Here's how the part is built. I have some questions about the finished solid (model axes, mm). A direction names the side the tool comes from. Give positions to 0.01 mm unless a question says otherwise; leave off trailing zeros. Loops run counter-clockwise (first coordinate to the right, second up) from the corner with the lowest first, then second, coordinate; pieces in that order, holes last. Notation, with made-up numbers: M 58,56.25 L 108,56.25 A20 ccw 108,66.25 Z; hole C 0.25,9.5 d2. An arc over 180 degrees is marked long. Answer as CSV lines item,"result". Start each with the question number.
Item 1: For faces 1 (the flat face through (4.661, 49, 25)), 2 (the flat face through (54, 10, 15)), 3 (the flat face through (100, 5, 15)), which set-ups out of +Z, -Z, +X, -X, +Y, -Y let a thin tool reach every point of the face, with its end or its side?
Item 2: I want a section at B-B on z = 12.5. List the corners of the cut face in (x, y) for me, plus the area to 3 significant figures.
Item 3: I want a section at C-C on z = 5. List the corners of the cut face in (x, y) for me.
Item 4: If we mould it in two halves opening along Z, with no side actions, what happens to faces 4 (the flat face through (31, 9, 30)), 5 (the flat face through (6, 54, 11)), 6 (the cylindrical face through (4.023, 75.483, 12.24)), 7 (the cylindrical face through (4.023, 37.548, 12.066))? For each: released by +Z, released by -Z, zero draft, split by the parting line, or undercut.
Item 5: Will these pins go through, and if not, where does the flat tip stop? P1, Ø3, axis at y = 54, z = 25, coming from the +X side; P2, Ø1.1, axis at x = 5.5, y = 44, coming from the +Z side; P3, Ø9, axis at y = 33.5, z = 8.5, coming from the +X side; P4, Ø1, axis at x = 46.5, z = 9, coming from the -Y side.
Item 6: I want a section at D-D on y = 39.5. List the corners of the cut face in (x, z) for me, plus the area to 3 significant figures.
Item 7: If I drill on line 1 along Y through (x, z) = (4.05, 12.5); line 2 along Y through (x, z) = (21.5, 24); line 3 along X through (y, z) = (72.5, 5.5), over which ranges is the centre line in solid material (lowest first)? Write a range as from..to.
Item 8: I want a section at A-A on y = 73.5. List the corners of the cut face in (x, z) for me, plus the area to 3 significant figures.
from build123d import *

# Parameters (mm, degrees)
BOSS_EXTRUDE1_DEPTH = 30
SKETCH2_R           = 2
CUT_EXTRUDE1_DEPTH  = 145.568322948
CHAMFER1_SIZE       = 2.1
SKETCH3_W           = 2.678240958
SKETCH3_H           = 39.075972863
CUT_EXTRUDE2_DEPTH  = 10


with BuildPart() as part:
    # Sketch1 → Boss-Extrude1 (new body)
    with BuildSketch(Plane.XY):
        Polygon((0, 0), (100, 0), (100, 10), (6, 10), (6, 100), (0, 100), align=None)
    extrude(amount=BOSS_EXTRUDE1_DEPTH)

    # Sketch2 → Cut-Extrude1 (cut, through all)
    with BuildSketch(Plane.ZY):
        with Locations((12.5, 73.5)):
            Circle(SKETCH2_R)
        with Locations((12.5, 39.5)):
            Circle(SKETCH2_R)
    extrude(amount=-CUT_EXTRUDE1_DEPTH, mode=Mode.SUBTRACT)

    # Chamfer1
    chamfer1_edges = [part.edges().sort_by_distance(p)[0] for p in [
        (0, 73.5, 10.5),
        (0, 39.5, 10.5),
    ]]
    chamfer(chamfer1_edges, length=CHAMFER1_SIZE)

    # Sketch3 → Cut-Extrude2 (cut)
    with BuildSketch(Plane.XY.offset(30)):
        with Locations((6, 49.716029753)):
            Rectangle(SKETCH3_W, SKETCH3_H)
    extrude(amount=-CUT_EXTRUDE2_DEPTH, mode=Mode.SUBTRACT)


solid = part.part
Result:
1,face 1,"+Z, +X"
1,face 2,"+Z, -Z, +X, +Y"
1,face 3,"+Z, -Z, +X, +Y, -Y"
2,outline,"M 0,0 L 100,0 L 100,10 L 6,10 L 6,37.5 L 2.1,37.5 L 0,35.4 Z; M 0,43.6 L 2.1,41.5 L 6,41.5 L 6,71.5 L 2.1,71.5 L 0,69.4 Z; M 0,77.6 L 2.1,75.5 L 6,75.5 L 6,100 L 0,100 Z"
2,area,"1,480 mm^2"
3,outline,"M 0,0 L 100,0 L 100,10 L 6,10 L 6,100 L 0,100 Z"
4,face 4,"released by +Z"
4,face 5,"zero draft"
4,face 6,"undercut"
4,face 7,"undercut"
5,P1,"x = 4.66"
5,P2,"z = 20"
5,P3,"x = 6"
5,P4,"y = 0"
6,outline,"M 0,0 L 6,0 L 6,10.5 L 2.1,10.5 L 0,8.4 Z; M 0,16.6 L 2.1,14.5 L 6,14.5 L 6,20 L 4.66,20 L 4.66,30 L 0,30 Z"
6,area,"138 mm^2"
7,line 1,"0..37.5, 41.5..71.5, 75.5..100"
7,line 2,"0..10"
7,line 3,"0..6"
8,outline,"M 0,0 L 6,0 L 6,10.5 L 2.1,10.5 L 0,8.4 Z; M 0,16.6 L 2.1,14.5 L 6,14.5 L 6,30 L 0,30 Z"
8,area,"152 mm^2"
